from build123d import *

# Parameters (mm, degrees)
EXTRUDE_THIN_2_DEPTH = 2.18


with BuildPart() as part:
    # Sketch 1 → Extrude-thin 2 (new body)
    with BuildSketch(Plane(origin=(0, 0, 0), x_dir=(1, 0, 0), z_dir=(0, 1, 0))):
        with BuildLine():
            ThreePointArc((0, -2.5), (2.5, 0), (0, 2.5))
            ThreePointArc((0, 2.5), (-3.4375, -0.9375), (0, -4.375))
            ThreePointArc((0, -4.375), (4.375, 0), (0, 4.375))
            ThreePointArc((0, 4.375), (-5.3125, -0.9375), (0, -6.25))
            ThreePointArc((0, -6.25), (6.25, 0), (0, 6.25))
            ThreePointArc((0, 6.25), (-7.1875, -0.9375), (0, -8.125))
            ThreePointArc((0, -8.125), (8.125, 0), (0, 8.125))
            ThreePointArc((0, 8.125), (-9.0625, -0.9375), (0, -10))
            ThreePointArc((0, -10), (10, 0), (0, 10))
            ThreePointArc((0, 10), (-10.9375, -0.9375), (0, -11.875))
            ThreePointArc((0, -11.875), (11.875, 0), (0, 11.875))
            ThreePointArc((0, 11.875), (-12.8125, -0.9375), (0, -13.75))
            ThreePointArc((0, -13.75), (13.75, 0), (0, 13.75))
            ThreePointArc((0, 13.75), (-14.6875, -0.9375), (0, -15.625))
            ThreePointArc((0, -15.625), (15.625, 0), (0, 15.625))
            ThreePointArc((0, 15.625), (-16.5625, -0.9375), (0, -17.5))
            ThreePointArc((0, -17.5), (17.5, 0), (0, 17.5))
            Line((0, 17.5), (0, 17.86))
            ThreePointArc((0, 17.86), (17.86, 0), (0, -17.86))
            ThreePointArc((0, -17.86), (-16.9225, -0.9375), (0, 15.985))
            ThreePointArc((0, 15.985), (15.985, 0), (0, -15.985))
            ThreePointArc((0, -15.985), (-15.0475, -0.9375), (0, 14.11))
            ThreePointArc((0, 14.11), (14.11, 0), (0, -14.11))
            ThreePointArc((0, -14.11), (-13.1725, -0.9375), (0, 12.235))
            ThreePointArc((0, 12.235), (12.235, 0), (0, -12.235))
            ThreePointArc((0, -12.235), (-11.2975, -0.9375), (0, 10.36))
            ThreePointArc((0, 10.36), (10.36, 0), (0, -10.36))
            ThreePointArc((0, -10.36), (-9.4225, -0.9375), (0, 8.485))
            ThreePointArc((0, 8.485), (8.485, 0), (0, -8.485))
            ThreePointArc((0, -8.485), (-7.5475, -0.9375), (0, 6.61))
            ThreePointArc((0, 6.61), (6.61, 0), (0, -6.61))
            ThreePointArc((0, -6.61), (-5.6725, -0.9375), (0, 4.735))
            ThreePointArc((0, 4.735), (4.735, 0), (0, -4.735))
            ThreePointArc((0, -4.735), (-3.7975, -0.9375), (0, 2.86))
            ThreePointArc((0, 2.86), (2.86, 0), (0, -2.86))
            Line((0, -2.86), (0, -2.5))
        make_face()
    extrude(amount=EXTRUDE_THIN_2_DEPTH)


solid = part.part
The model under review builds one solid part; all positions refer to its coordinate system, in mm. Coordinates: 2 decimals unless noted, no trailing zeros.
(1) Wall thickness on L1, parallel to Z at x = 12.5, y = 0.6 (3 decimals): over which ranges is the line inside the solid? List them lowest first.
Determined:
L1: z = -12.757 to -12.247, -9.963 to -9.375, -6.545 to -5.728, 5.728 to 6.545, 9.375 to 9.963, 12.247 to 12.757
(2) Draft analysis for pull direction X (two halves, no side actions). For faces 1 (the flat face through (-3, 2.18, 3)), 2 (the cylindrical face through (2.5, 1.1, 0.1)), state which applies: +X half, -X half, draft (parallel to the pull), parting line (faces both ways), or undercut.
Determined:
face 1: draft
face 2: undercut
(3) Insertion check: P1, Ø1, axis at x = -6, z = 4.5, coming from the +Y side. The pin has a flat end and moves straight along its axis. Give the tip position at first contact, or say it passes through.
Determined:
P1: stops at y = 2.18
(4) Consider section A-A, the plane x = 11. Give the number of separate pieces and of enclosed holes in the cut face, plus the area to 3 significant figures.
Determined:
separate pieces: 8
enclosed holes: 0
area: 10.6 mm2
